```python
from build123d import *

# Parameters (mm, degrees)
EXTRUDE_1_DEPTH = 800


with BuildPart() as part:
    # 草图1 → 凸台-拉伸1 (new body)
    with BuildSketch(Plane.XY):
        Polygon((-10, -12.5), (-14, -12.5), (-14, -65.5), (11, -65.5), (11, -15.5), (-10, -15.5), align=None)
    extrude(amount=-EXTRUDE_1_DEPTH)


solid = part.part
```
Can you work these out from the model? Positions are in its coordinate system, mm. A direction names the side the tool comes from. Round coordinates to 2 decimals unless told otherwise and drop trailing zeros. Loops run counter-clockwise (first coordinate to the right, second up) from the corner with the lowest first, then second, coordinate; pieces in that order, holes last. Notation, with made-up numbers: M 83,76.5 L 100,76.5 A23 cw 100,103.5 Z; hole C -27.75,7 d1. An arc over 180 degrees is marked long. Write item = value, one per line. Start each with the question number.
(1) Which directions (+Z, -Z, +X, -X, +Y, -Y) give clear straight access to the entire face, cutting with the end or side of a thin tool? Please do faces 1 (the face through (-2, -39, 0)), 2 (the face through (1, -15.5, -394)).
(2) I need wall thicknesses on line 1 along Y through (x, z) = (1.5, -277). Which ranges of the line are inside material? Lowest first, please.
(3) Suppose I cut it at A-A on z = -150.5. Write out the boundary of the cut face in (x, y).
(4) I'm going to push flat-ended pins straight in: P1, Ø10, axis at x = -6.5, y = -31, coming from the +Z side; P2, Ø0.9, axis at y = -14.5, z = -554.5, coming from the +X side. Where does each tip first touch, or does it pass through?
(5) Suppose I cut it at B-B on x = 6.75. Write out the boundary of the cut face in (y, z).
Answer block:
q1.face_1 = +Z, +X, -X, +Y, -Y
q1.face_2 = +Z, -Z, +X, +Y
q2.line_1 = -65.5 to -15.5
q3.outline = M -14,-65.5 L 11,-65.5 L 11,-15.5 L -10,-15.5 L -10,-12.5 L -14,-12.5 Z
q4.P1 = 0
q4.P2 = -10
q5.outline = M -65.5,-800 L -15.5,-800 L -15.5,0 L -65.5,0 Z
